from build123d import *

# Parameters (mm, degrees)
SKETCH1_W           = 175
SKETCH1_H           = 63
BOSS_EXTRUDE1_DEPTH = 5
CUT_EXTRUDE1_DEPTH  = 5
CHAMFER1_SIZE       = 15
CHAMFER2_SIZE       = 5
BOSS_EXTRUDE2_START = -7
BOSS_EXTRUDE2_DEPTH = 25
SKETCH4_W           = 68
SKETCH4_H           = 5
SKETCH4_W_2         = 70
BOSS_EXTRUDE3_DEPTH = 2


with BuildPart() as part:
    # Sketch1 → Boss-Extrude1 (new body)
    with BuildSketch(Plane.XY):
        with Locations((0, 24.5)):
            Rectangle(SKETCH1_W, SKETCH1_H)
    extrude(amount=BOSS_EXTRUDE1_DEPTH)

    # Sketch2 → Cut-Extrude1 (cut)
    with BuildSketch(Plane.XY.offset(5)):
        Polygon((-74.5, 56), (-4.5, 56), (-4.5, 43.378679656), (-10.378679656, 37.5), (-68.621320344, 37.5), (-74.5, 43.378679656), align=None)
    extrude(amount=-CUT_EXTRUDE1_DEPTH, mode=Mode.SUBTRACT)

    # Chamfer1
    chamfer1_edges = [part.edges().sort_by_distance(p)[0] for p in [
        (87.5, -7, 2.5),
        (-87.5, -7, 2.5),
    ]]
    chamfer(chamfer1_edges, length=CHAMFER1_SIZE)

    # Chamfer2
    chamfer2_edges = [part.edges().sort_by_distance(p)[0] for p in [
        (-87.5, 56, 2.5),
        (87.5, 56, 2.5),
    ]]
    chamfer(chamfer2_edges, length=CHAMFER2_SIZE)

    # Sketch3 → Boss-Extrude2 (add)
    with BuildSketch(Plane.XZ.offset(7).offset(BOSS_EXTRUDE2_START)):
        Polygon((51.767949192, 0), (25.232050808, 0), (23.5, -3), (53.5, -3), align=None)
        Polygon((-53.5, -3), (-23.5, -3), (-25.232050808, 0), (-51.767949192, 0), align=None)
    extrude(amount=-BOSS_EXTRUDE2_DEPTH)

    # Sketch4 → Boss-Extrude3 (add)
    with BuildSketch(Plane(origin=(0, 25, 0), x_dir=(1, 0, 0), z_dir=(0, 1, 0))):
        with Locations((-39.5, 2.5)):
            Rectangle(SKETCH4_W, SKETCH4_H)
        with Locations((38.5, 2.5)):
            Rectangle(SKETCH4_W_2, SKETCH4_H)
    extrude(amount=-BOSS_EXTRUDE3_DEPTH)


solid = part.part
Could you check a few things on this model? Use its own coordinates, in mm. A direction names the side the tool comes from. Give positions to 0.01 mm unless a question says otherwise; leave off trailing zeros. Order: outer loops, then holes, each group sorted by start corner. A loop starts at its lowest first (then second) coordinate and runs counter-clockwise, first axis right, second up. Notation, with made-up numbers: (-14.5, 77) -> (37.5, 77) arc R24 ccw to (37.5, 110) -> close; hole circle Ø8 at (35.5, 63.25). An arc over 180 degrees is marked (long way). Return JSON: item names as keys, results as strings.
1. Imagine slicing it at A-A on y = 49.5. List the corners of the cut face in (x, z) for me, then the cut area to 3 significant figures.
Answer list:
{"outline": "(-87.5, 0) -> (-74.5, 0) -> (-74.5, 5) -> (-87.5, 5) -> close; (-4.5, 0) -> (87.5, 0) -> (87.5, 5) -> (-4.5, 5) -> close", "area": "525 mm2"}
2. On a 3-axis mill with a long thin cutter (end or side, diameter ignored), from which of +Z, -Z, +X, -X, +Y, -Y can I reach the whole of each face in a straight line? I mean faces 4 (the flat face through (87.5, 29, 2)), 5 (the flat face through (-74.5, 50, 3)), 6 (the flat face through (38, 0, -1)). Say none if no direction works.
Answer list:
{"face 4": "+Z, -Z, +X, +Y, -Y", "face 5": "+Z, -Z, +Y", "face 6": "-Z, +X, -X, -Y"}
3. I need wall thicknesses on line 1 (Z direction, x = -55.5, y = 18); line 2 (X direction, y = 11, z = -0.5); line 3 (Y direction, x = -51, z = -2). Which ranges of each line are inside material? Lowest first, please. Write a range as from..to.
Answer list:
{"line 1": "z = 0..5", "line 2": "x = -52.06..-24.94, 24.94..52.06", "line 3": "y = 0..25"}
4. Imagine slicing it at C-C on z = 3. List the corners of the cut face in (x, y) for me.
Answer list:
{"outline": "(-87.5, 8) -> (-72.5, -7) -> (72.5, -7) -> (87.5, 8) -> (87.5, 51) -> (82.5, 56) -> (-4.5, 56) -> (-4.5, 43.38) -> (-10.38, 37.5) -> (-68.62, 37.5) -> (-74.5, 43.38) -> (-74.5, 56) -> (-82.5, 56) -> (-87.5, 51) -> close"}
5. Thinking about a two-plate mould opening in Z: for faces 1 (the flat face through (-71.52, 40.4, 2.54)), 2 (the flat face through (24.378, 11.339, -1.479)), 3 (the flat face through (38, 11, -3)), which applies, pulls with the +Z half, pulls with the -Z half, needs draft (parallel to the pull), parting line crosses it, or undercut?
Answer list:
{"face 1": "needs draft", "face 2": "undercut", "face 3": "pulls with the -Z half"}
6. Imagine slicing it at B-B on x = 45. List the corners of the cut face in (y, z) for me.
Answer list:
{"outline": "(-7, 0) -> (0, 0) -> (0, -3) -> (23, -3) -> (23, -5) -> (25, -5) -> (25, 0) -> (56, 0) -> (56, 5) -> (-7, 5) -> close"}
7. Imagine slicing it at D-D on y = 4. List the corners of the cut face in (x, z) for me.
Answer list:
{"outline": "(-83.5, 0) -> (-51.77, 0) -> (-53.5, -3) -> (-23.5, -3) -> (-25.23, 0) -> (25.23, 0) -> (23.5, -3) -> (53.5, -3) -> (51.77, 0) -> (83.5, 0) -> (83.5, 5) -> (-83.5, 5) -> close"}
8. For pin 1 Ø1.6 at (y, z) = (24, -3) entering from -X; pin 2 Ø2.5 at (x, z) = (-51.5, -2.5) entering from -Y; pin 3 Ø1.5 at (y, z) = (52.5, 3) entering from -X, each with a flat end and sliding along its axis, tell me the tip position at first contact or that it passes through.
Answer list:
{"pin 1": "stops at x = -73.5", "pin 2": "stops at y = 0", "pin 3": "stops at x = -86.75"}
